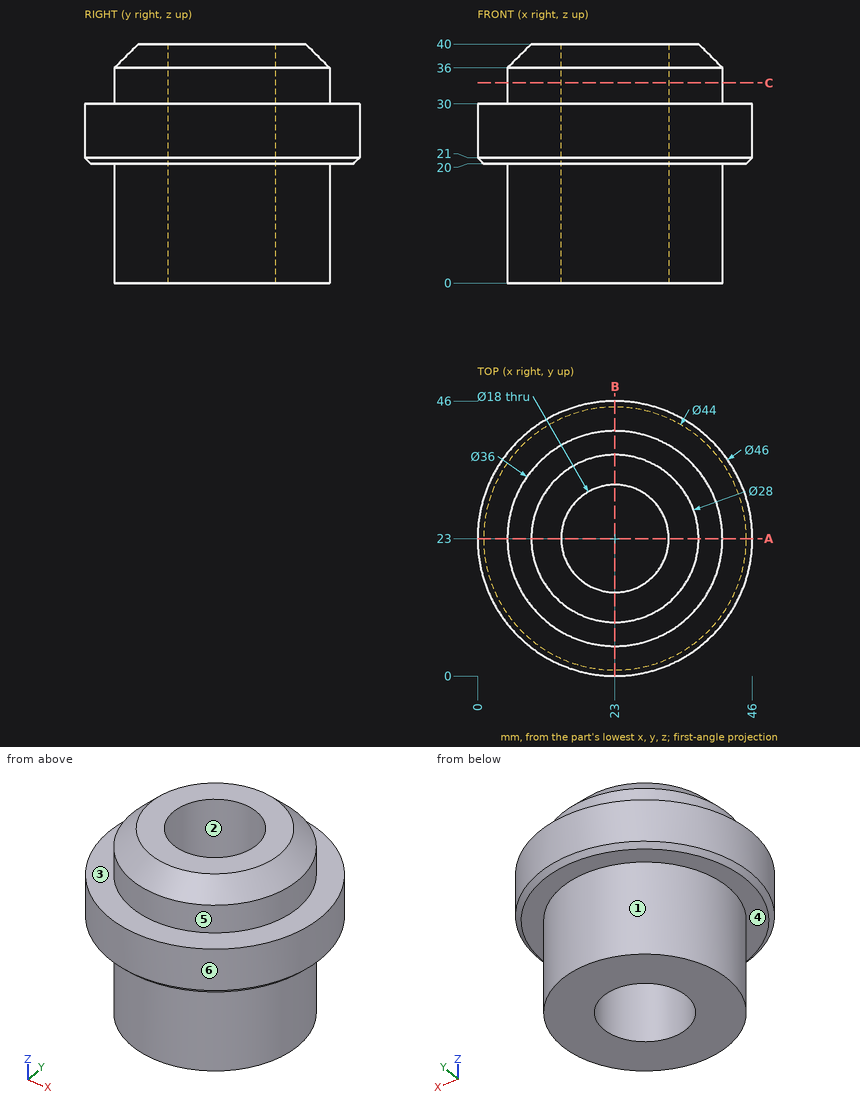
Check sheet for the drawn part. Datum: minimum x, y, z corner. Units: mm. A direction names the side the tool comes from. Round coordinates to 2 decimals unless told otherwise and drop trailing zeros. Order: outer loops, then holes, each group sorted by start corner. A loop starts at its lowest first (then second) coordinate and runs counter-clockwise, first axis right, second up. Notation, with made-up numbers: (37, 41) - (79, 41) arc R24 ccw to (79, 52) - close; hole circle Ø3 at (19, -3). An arc over 180 degrees is marked (long way). Use a Markdown table: item, result. Add a question column.
(1) Tool access check on the marked faces 4, 5 and 6. Record the directions out of +Z, -Z, +X, -X, +Y, -Y that give a thin tool (end or side, any length) a straight path to the whole face; none if there is none.
(2) Release check for a two-part mould opening along Y. For the marked faces 1, 2 and 3 record: pulls with the +Y half, pulls with the -Y half, needs draft (parallel to the pull), parting line crosses it, or undercut.
(3) Sectioned sample at C-C, the plane z = 33.5. Enter the section's corners in (x, y).
(4) Depth check by flat-ended pin: pin 1 (2 mm diameter, centred on x = 5.5, z = 27.5, fed in from +Y); pin 2 (12 mm diameter, centred on x = 21, z = 32.5, fed in from -Y); pin 3 (16 mm diameter, centred on x = 23, y = 23, fed in from -Z); pin 4 (8 mm diameter, centred on y = 37, z = 31.5, fed in from -X). Enter the tip coordinate at first touch or a pass-through.
(5) Material ranges on line 1 along Y through (x, z) = (23, 10); line 2 along Y through (x, z) = (23, 26); line 3 along Z through (x, y) = (8, 9.5), recorded low to high. Write a range as [from, to].
(6) Sectioned sample at A-A, the plane y = 23. Enter the section's corners in (x, z), and give its area (3 significant figures).
Answers below:
| question | item | result |
|---|---|---|
| 1 | face 4 | -Z |
| 1 | face 5 | +Z |
| 1 | face 6 | +Z, -Z |
| 2 | face 1 | parting line crosses it |
| 2 | face 2 | undercut |
| 2 | face 3 | needs draft |
| 3 | outline | circle Ø36 at (23, 23); hole circle Ø18 at (23, 23) |
| 4 | pin 1 | y = 39.02 |
| 4 | pin 2 | y = 0 |
| 4 | pin 3 | through |
| 4 | pin 4 | x = 2.43 |
| 5 | line 1 | [5, 14], [32, 41] |
| 5 | line 2 | [0, 14], [32, 46] |
| 5 | line 3 | [20, 30] |
| 6 | outline | (0, 21) - (1, 20) - (5, 20) - (5, 0) - (14, 0) - (14, 40) - (9, 40) - (5, 36) - (5, 30) - (0, 30) - close; (32, 0) - (41, 0) - (41, 20) - (45, 20) - (46, 21) - (46, 30) - (41, 30) - (41, 36) - (37, 40) - (32, 40) - close |
| 6 | area | 803 mm² |
